Geometry check sheet. Reference: the model listing, model coordinates, mm. Face numbers are marked on the shaded views. A direction names the side the tool comes from. Give positions to 0.01 mm unless a question says otherwise; leave off trailing zeros. Loops run counter-clockwise (first coordinate to the right, second up) from the corner with the lowest first, then second, coordinate; pieces in that order, holes last.
1. Material ranges on L1, parallel to X at y = 13, z = 0; L2, parallel to X at y = -20, z = -7.5; L3, parallel to Z at x = -81, y = 34, recorded low to high.
2. Release check for a two-part mould opening along X. For the marked faces 1 and 2 record: +X half, -X half, draft (parallel to the pull), parting line (faces both ways), or undercut.
3. Cross-section at D-D, the plane x = 19. Record the cut outline in (y, z).
4. Cross-section at A-A, the plane y = -52. State how many separate pieces and enclosed holes the cut face has, plus the area to 3 significant figures.
5. Go/stop test with flat-tipped pins: pin 1 Ø2.5 at (x, z) = (-54.5, 0.5) entering from +Y; pin 2 Ø15 at (x, z) = (-12.5, 26) entering from -Y. Record where each tip stops, or that it passes through.
6. Cross-section at C-C, the plane y = -27. Record the cut outline in (x, z), plus the area to 3 significant figures.
7. Tool access check on the marked faces 3, 4 and 5. Record the directions out of +Z, -Z, +X, -X, +Y, -Y that give a thin tool (end or side, any length) a straight path to the whole face; none if there is none.
8. Cross-section at B-B, the plane z = 0. Record the cut outline in (x, y).
from build123d import *

# Parameters (mm, degrees)
BLOCK_BODY_DEPTH             = 45.5
CRANKSHAFT_BORE_SKETCH_R     = 17.5
CRANKSHAFT_BORE_35_DEPTH     = 265.547727263
CYLINDER_BORES_SKETCH_R      = 30.05
CYLINDER_BORES_3X_45_5_DEPTH = 81


with BuildPart() as part:
    # Block Profile Sketch → Block Body (new, symmetric)
    with BuildSketch(Plane.XY):
        Polygon((-106.5, -62.5), (-106.5, 2.5), (-55.5, 2.5), (-55.5, -62.5), (-25.5, -62.5), (-25.5, 2.5), (25.5, 2.5), (25.5, -62.5), (55.5, -62.5), (55.5, 2.5), (106.5, 2.5), (106.5, -62.5), (126.5, -62.5), (126.5, 62.5), (-126.5, 62.5), (-126.5, -62.5), align=None)
    extrude(amount=BLOCK_BODY_DEPTH, both=True)

    # Crankshaft Bore Sketch → Crankshaft Bore Ø35 (cut, through all)
    with BuildSketch(Plane(origin=(126.5, 0, 0), x_dir=(0, 0, -1), z_dir=(1, 0, 0))):
        with Locations((0, -62.5)):
            Circle(CRANKSHAFT_BORE_SKETCH_R)
    extrude(amount=-CRANKSHAFT_BORE_35_DEPTH, mode=Mode.SUBTRACT)

    # Cylinder Bores Sketch → Cylinder Bores 3xØ45.5 (cut)
    with BuildSketch(Plane(origin=(0, 62.5, 0), x_dir=(1, 0, 0), z_dir=(0, 1, 0))):
        with Locations(Location((-81, 0, 0), (0, 0, 270))):
            Circle(CYLINDER_BORES_SKETCH_R)
        with Locations(Location((0, 0, 0), (0, 0, 270))):
            Circle(CYLINDER_BORES_SKETCH_R)
        with Locations(Location((81, 0, 0), (0, 0, 270))):
            Circle(CYLINDER_BORES_SKETCH_R)
    extrude(amount=-CYLINDER_BORES_3X_45_5_DEPTH, mode=Mode.SUBTRACT)


solid = part.part
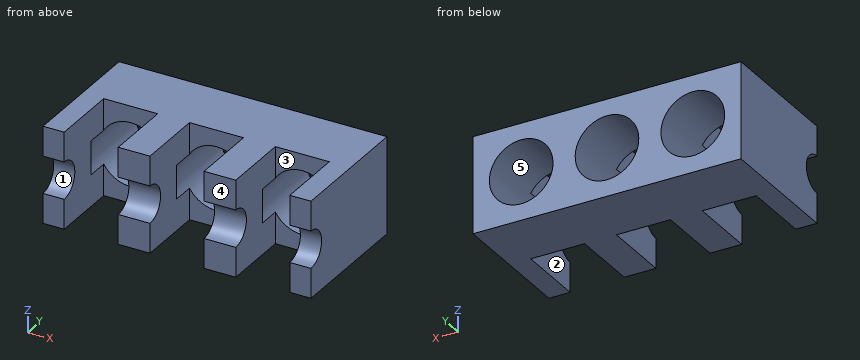
Result:
1. L1: x = -126.5 to -111.05, -50.95 to -30.05, 30.05 to 50.95, 111.05 to 126.5
1. L2: x = -126.5 to -106.5, -55.5 to -25.5, 25.5 to 55.5, 106.5 to 126.5
1. L3: z = -45.5 to -30.05, 30.05 to 45.5
2. face 1: draft
2. face 2: undercut
3. outline: (2.5, -45.5) - (62.5, -45.5) - (62.5, -23.28) - (2.5, -23.28) - close; (2.5, 23.28) - (62.5, 23.28) - (62.5, 45.5) - (2.5, 45.5) - close
4. separate pieces: 8
4. enclosed holes: 0
4. area: 6,300 mm2
5. pin 1: stops at y = -18.5
5. pin 2: stops at y = 2.5
6. outline: (-126.5, -45.5) - (-106.5, -45.5) - (-106.5, 45.5) - (-126.5, 45.5) - close; (-55.5, -45.5) - (-25.5, -45.5) - (-25.5, 45.5) - (-55.5, 45.5) - close; (25.5, -45.5) - (55.5, -45.5) - (55.5, 45.5) - (25.5, 45.5) - close; (106.5, -45.5) - (126.5, -45.5) - (126.5, 45.5) - (106.5, 45.5) - close
6. area: 9,100 mm2
7. face 3: +Z, -Z, -Y
7. face 4: +Z, -Z, +X, -X, -Y
7. face 5: +Y
8. outline: (-126.5, -45) - (-106.5, -45) - (-106.5, -18.5) - (-111.05, -18.5) - (-111.05, 62.5) - (-126.5, 62.5) - close; (-55.5, -45) - (-25.5, -45) - (-25.5, -18.5) - (-30.05, -18.5) - (-30.05, 62.5) - (-50.95, 62.5) - (-50.95, -18.5) - (-55.5, -18.5) - close; (25.5, -45) - (55.5, -45) - (55.5, -18.5) - (50.95, -18.5) - (50.95, 62.5) - (30.05, 62.5) - (30.05, -18.5) - (25.5, -18.5) - close; (106.5, -45) - (126.5, -45) - (126.5, 62.5) - (111.05, 62.5) - (111.05, -18.5) - (106.5, -18.5) - close
